```python
from build123d import *

# Parameters (mm, degrees)
SKETCH1_W               = 400
SKETCH1_H               = 400
SKETCH1_R               = 2.5
BOSS_EXTRUDE1_DEPTH     = 5
SKETCH4_R               = 5
CUT_EXTRUDE1_DEPTH      = 283.886903196
SKETCH6_W               = 6
SKETCH6_H               = 10
BOSS_EXTRUDE4_DEPTH     = 26
CUT_EXTRUDE2_DEPTH      = 348.922405142
CUT_EXTRUDE2_DEPTH_BACK = 348.922405142
SKETCH8_W               = 5
SKETCH8_H               = 5
SKETCH9_W               = 10
SKETCH9_H               = 6
BOSS_EXTRUDE5_DEPTH     = 19
CUT_EXTRUDE3_DEPTH      = 328.123829765
CUT_EXTRUDE3_DEPTH_BACK = 328.123829765
SKETCH10_W              = 5
SKETCH10_H              = 5
SKETCH11_R              = 5.5
BOSS_EXTRUDE7_DEPTH     = 29


with BuildPart() as part:
    # Sketch1 → Boss-Extrude1 (new body)
    with BuildSketch(Plane.XY):
        Rectangle(SKETCH1_W, SKETCH1_H)
        with Locations((0, 10)):
            Circle(SKETCH1_R, mode=Mode.SUBTRACT)
        with Locations((80, 10)):
            Circle(SKETCH1_R, mode=Mode.SUBTRACT)
        with Locations((150, 180)):
            Circle(SKETCH1_R, mode=Mode.SUBTRACT)
        with Locations((150, 60)):
            Circle(SKETCH1_R, mode=Mode.SUBTRACT)
    extrude(amount=BOSS_EXTRUDE1_DEPTH)

    # Sketch4 → Cut-Extrude1 (cut, through all)
    with BuildSketch(Plane.XY.offset(5)):
        with Locations((-125, 10)):
            Circle(SKETCH4_R)
        with Locations((150, -125)):
            Circle(SKETCH4_R)
    extrude(amount=-CUT_EXTRUDE1_DEPTH, mode=Mode.SUBTRACT)

    # Sketch6 → Boss-Extrude4 (add)
    with BuildSketch(Plane.XY.offset(5)):
        with Locations((0, 10)):
            Rectangle(SKETCH6_W, SKETCH6_H)
        with Locations((80, 10)):
            Rectangle(SKETCH6_W, SKETCH6_H)
    extrude(amount=BOSS_EXTRUDE4_DEPTH)

    # Sketch8 → Cut-Extrude2 (cut, two sides: drawn at the far end of the back side and taken through both)
    with BuildSketch(Plane(origin=(83, 0, 0), x_dir=(0, 0, -1), z_dir=(1, 0, 0)).offset(-CUT_EXTRUDE2_DEPTH_BACK)):
        with Locations((-26, 10)):
            Rectangle(SKETCH8_W, SKETCH8_H)
    extrude(amount=CUT_EXTRUDE2_DEPTH + CUT_EXTRUDE2_DEPTH_BACK, mode=Mode.SUBTRACT)

    # Sketch9 → Boss-Extrude5 (add)
    with BuildSketch(Plane.XY.offset(5)):
        with Locations((150, 180)):
            Rectangle(SKETCH9_W, SKETCH9_H)
        with Locations((150, 60)):
            Rectangle(SKETCH9_W, SKETCH9_H)
    extrude(amount=BOSS_EXTRUDE5_DEPTH)

    # Sketch10 → Cut-Extrude3 (cut, two sides: drawn at the far end of the back side and taken through both)
    with BuildSketch(Plane(origin=(0, 57, 0), x_dir=(-1, 0, 0), z_dir=(0, -1, 0)).offset(-CUT_EXTRUDE3_DEPTH_BACK)):
        with Locations((-150, -19)):
            Rectangle(SKETCH10_W, SKETCH10_H)
    extrude(amount=CUT_EXTRUDE3_DEPTH + CUT_EXTRUDE3_DEPTH_BACK, mode=Mode.SUBTRACT)

    # Sketch11 → Boss-Extrude7 (add)
    with BuildSketch(Plane.XY.offset(5)):
        with Locations((-125, 10)):
            Circle(SKETCH11_R)
        with Locations((150, -125)):
            Circle(SKETCH11_R)
    extrude(amount=BOSS_EXTRUDE7_DEPTH)


solid = part.part
```
Check sheet for the modelled part. Datum: model origin and axes. Units: mm. A direction names the side the tool comes from. Coordinates: 2 decimals unless noted, no trailing zeros. Order: outer loops, then holes, each group sorted by start corner. A loop starts at its lowest first (then second) coordinate and runs counter-clockwise, first axis right, second up. Notation, with made-up numbers: (-26, 63) -> (1, 63) arc R14 ccw to (1, 75) -> close; hole circle Ø6 at (44.5, 41). An arc over 180 degrees is marked (long way). Write each question's results on one line, items separated by ' | '. Start each with the question number.
1) Section check C-C (x = 109.5). Enter the section's corners in (y, z).
2) Draft check along Y on faces 4 (the face through (-3, 10, 18)), 5 (the face through (150, 57, 14)), 6 (the face through (150, 183, 14)). Enter one of: pulls with the +Y half, pulls with the -Y half, needs draft (parallel to the pull), parting line crosses it, or undercut.
3) Depth check by flat-ended pin: pin 1 (10 mm diameter, centred on x = -40, y = 129.5, fed in from +Z); pin 2 (11 mm diameter, centred on x = 150, y = -127, fed in from -Z); pin 3 (1.5 mm diameter, centred on x = 150.5, y = 59, fed in from +Z); pin 4 (1.8 mm diameter, centred on y = 60.5, z = 17, fed in from -X). Enter the tip coordinate at first touch or a pass-through.
4) Set-up check for faces 1 (the face through (149.284, -119.547, 19.297)), 2 (the face through (-120.381, 8.085, 2.535)), 3 (the face through (77, 10, 18)): record each of +Z, -Z, +X, -X, +Y, -Y from which the full face is reachable in a straight line by a thin tool's end or side.
5) Section check B-B (y = -125). Enter the section's corners in (x, z), and give its area (3 significant figures).
6) Material ranges on line 1 along Z through (x, y) = (-118, 92); line 2 along Y through (x, z) = (-125, 3.55), recorded low to high.
7) Section check A-A (z = 11). Enter the section's corners in (x, y).
Checked values:
1) outline: (-200, 0) -> (200, 0) -> (200, 5) -> (-200, 5) -> close
2) face 4: needs draft | face 5: undercut | face 6: pulls with the +Y half
3) pin 1: z = 5 | pin 2: z = 0 | pin 3: z = 24 | pin 4: x = 145
4) face 1: +Z | face 2: -Z | face 3: +Z, +Y, -Y
5) outline: (-200, 0) -> (145, 0) -> (145, 5) -> (155, 5) -> (155, 0) -> (200, 0) -> (200, 5) -> (155.5, 5) -> (155.5, 34) -> (144.5, 34) -> (144.5, 5) -> (-200, 5) -> close | area: 2,270 mm²
6) line 1: 0 to 5 | line 2: -200 to 5, 15 to 200
7) outline: circle Ø11 at (-125, 10); (-3, 5) -> (3, 5) -> (3, 15) -> (-3, 15) -> close; (77, 5) -> (83, 5) -> (83, 15) -> (77, 15) -> close; circle Ø11 at (150, -125); (145, 57) -> (155, 57) -> (155, 63) -> (145, 63) -> close; (145, 177) -> (155, 177) -> (155, 183) -> (145, 183) -> close
